from build123d import *

# Parameters (mm, degrees)
BOSS_EXTRUDE1_DEPTH = 200
SKETCH2_W           = 63
SKETCH2_H           = 196
CUT_EXTRUDE1_DEPTH  = 17
SKETCH3_W           = 67
SKETCH3_H           = 17
BOSS_EXTRUDE2_DEPTH = 5
CHAMFER1_SIZE       = 5


with BuildPart() as part:
    # Sketch1 → Boss-Extrude1 (new body)
    with BuildSketch(Plane.XY):
        Polygon((-73, 28), (-6, 28), (-6, 32.656854249), (-1, 37.656854249), (-1, 39.353196257), (-6, 44.353196257), (-6, 47), (-73, 47), (-73, 44.353196257), (-78, 39.353196257), (-78, 37.656854249), (-73, 32.656854249), align=None)
    extrude(amount=-BOSS_EXTRUDE1_DEPTH)

    # Sketch2 → Cut-Extrude1 (cut)
    with BuildSketch(Plane(origin=(0, 47, 0), x_dir=(1, 0, 0), z_dir=(0, 1, 0))):
        with Locations((-39.5, 100)):
            Rectangle(SKETCH2_W, SKETCH2_H)
    extrude(amount=-CUT_EXTRUDE1_DEPTH, mode=Mode.SUBTRACT)

    # Sketch3 → Boss-Extrude2 (add)
    with BuildSketch(Plane.XY):
        with Locations((-39.5, 47.5)):
            Rectangle(SKETCH3_W, SKETCH3_H)
    extrude(amount=BOSS_EXTRUDE2_DEPTH)

    # Chamfer1
    chamfer1_edges = [part.edges().sort_by_distance(p)[0] for p in [
        (-73, 39, 2.5),
        (-6, 39, 2.5),
    ]]
    chamfer(chamfer1_edges, length=CHAMFER1_SIZE)


solid = part.part
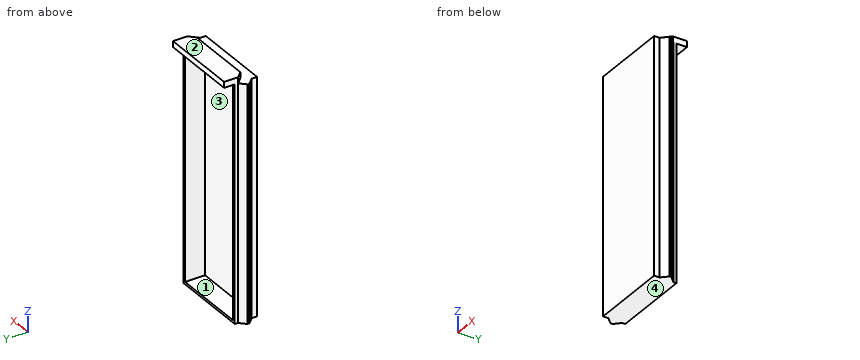
For this review, take the finished solid that the model builds, in its own axes (mm). Face numbers are marked on the shaded views. A direction names the side the tool comes from. Coordinates: 2 decimals unless noted, no trailing zeros. Order: outer loops, then holes, each group sorted by start corner. A loop starts at its lowest first (then second) coordinate and runs counter-clockwise, first axis right, second up. Notation, with made-up numbers: (9.5, 36.5) - (44.5, 36.5) arc R36 ccw to (44.5, 74.5) - close; hole circle Ø9 at (-18.5, -23). An arc over 180 degrees is marked (long way). Use one line per item in the form item = value.
Q1. For probe 1 along X at (y, z) = (32, -22); probe 2 along Z at (x, y) = (-23.5, 46.5); probe 3 along Z at (x, y) = (-22.5, 31), list the stretches that pass through material, from the lowest coordinate up. Write a range as from..to.
Checked values:
probe_1 = -73..-71, -8..-6
probe_2 = -200..-198, -2..5
probe_3 = -200..-198, -2..0
Q2. Consider section A-A (z = -134.5). Give the boundary of the cut face in (x, y).
Checked values:
outline = (-78, 37.66) - (-73, 32.66) - (-73, 28) - (-6, 28) - (-6, 32.66) - (-1, 37.66) - (-1, 39.35) - (-6, 44.35) - (-6, 47) - (-8, 47) - (-8, 30) - (-71, 30) - (-71, 47) - (-73, 47) - (-73, 44.35) - (-78, 39.35) - close
Q3. Consider section C-C (y = 41.5). Give the boundary of the cut face in (x, z).
Checked values:
outline = (-75.85, -200) - (-3.15, -200) - (-3.15, 0) - (-8.5, 0) - (-8.5, 5) - (-70.5, 5) - (-70.5, 0) - (-75.85, 0) - close; hole (-71, -198) - (-8, -198) - (-8, -2) - (-71, -2) - close
Q4. Consider section B-B (x = -60.5). Give the boundary of the cut face in (y, z).
Checked values:
outline = (28, -200) - (47, -200) - (47, -198) - (30, -198) - (30, -2) - (47, -2) - (47, 0) - (56, 0) - (56, 5) - (39, 5) - (39, 0) - (28, 0) - close
Q5. Consider section D-D (y = 50.5). Give the boundary of the cut face in (x, z), then the cut area to 3 significant figures.
Checked values:
outline = (-73, 0) - (-6, 0) - (-6, 5) - (-73, 5) - close
area = 335 mm2
Q6. For the marked faces 3 and 4, list the 3-axis set-ups (+Z, -Z, +X, -X, +Y, -Y) from which the entire face can be reached by the end or side of a thin tool; tool diameter is ignored.
Checked values:
face_3 = +Y
face_4 = -Z, +X, -X, +Y, -Y
Q7. Draft analysis for pull direction X (two halves, no side actions). For the marked faces 1 and 2, state which applies: +X half, -X half, draft (parallel to the pull), parting line (faces both ways), or undercut.
Checked values:
face_1 = undercut
face_2 = draft
Q8. For P1, Ø7, axis at x = -30.5, y = 51.5, coming from the -Z side; P2, Ø3, axis at x = -22.5, y = 34.5, coming from the +Z side; P3, Ø9.5, axis at y = 51, z = -124.5, coming from the +X side, all flat-tipped, find the tip position at first contact; note any pin that passes through.
Checked values:
P1 = 0
P2 = 0
P3 = -6
